```python
from build123d import *

# Parameters (mm, degrees)
BOSS_EXTRUDE1_DEPTH = 80
SKETCH2_R           = 6
CUT_EXTRUDE1_DEPTH  = 12


with BuildPart() as part:
    # Sketch1 → Boss-Extrude1 (new body)
    with BuildSketch(Plane.XY):
        with BuildLine():
            Line((0, 0), (-27, 0))
            ThreePointArc((-27, 0), (-36.192388155, -3.807611845), (-40, -13))
            Line((-40, -13), (-40, -190))
            Line((-40, -190), (-32, -190))
            Line((-32, -190), (-32, -13))
            ThreePointArc((-32, -13), (-30.535533906, -9.464466094), (-27, -8))
            Line((-27, -8), (0, -8))
            Line((0, -8), (0, 0))
        make_face()
    extrude(amount=BOSS_EXTRUDE1_DEPTH)

    # Sketch2 → Cut-Extrude1 (cut)
    with BuildSketch(Plane(origin=(0, 0, 0), x_dir=(1, 0, 0), z_dir=(0, 1, 0))):
        with Locations(Location((-15, -40, 0), (0, 0, 270))):
            Circle(SKETCH2_R)
        Polygon((-20, 0), (0, -30), (0, 0), align=None)
        Polygon((0, -50), (0, -80), (-20, -80), align=None)
    extrude(amount=-CUT_EXTRUDE1_DEPTH, mode=Mode.SUBTRACT)


solid = part.part
```
Geometry check sheet. Reference: the model listing, model coordinates, mm. A direction names the side the tool comes from. Give positions to 0.01 mm unless a question says otherwise; leave off trailing zeros. Loops run counter-clockwise (first coordinate to the right, second up) from the corner with the lowest first, then second, coordinate; pieces in that order, holes last. Notation, with made-up numbers: M 17.25,87 L 32.25,87 A28 ccw 32.25,126 Z; hole C 51,-2 d9. An arc over 180 degrees is marked long. Write item = value, one per line. Start each with the question number.
1. Draft check along X on faces 1 (the face through (-22, 0, 39)), 2 (the face through (-10.94, -3.94, 35.58)), 3 (the face through (-31, -10, 39)). Enter one of: +X half, -X half, draft (parallel to the pull), parting line (faces both ways), or undercut.
2. Thickness scan on probe 1 along Y at (x, z) = (-25, 37); probe 2 along X at (y, z) = (-94, 36.5); probe 3 along X at (y, z) = (-4.75, 40). Record the ranges inside material, lowest first.
3. Go/stop test with flat-tipped pins: P1, Ø8, axis at x = -11.5, z = 34.5, coming from the -Y side; P2, Ø5, axis at y = -49.5, z = 28, coming from the +X side; P3, Ø8, axis at x = -35.5, z = 36, coming from the +Y side. Record where each tip stops, or that it passes through.
4. Section check B-B, the plane x = -15. Enter the section's corners in (y, z).
5. Section check A-A, the plane z = 40. Enter the section's corners in (x, y), plus the area to 3 significant figures.
6. Tool access check on faces 4 (the face through (-10, -4, 15)), 5 (the face through (-23, -8, 39)). Record the directions out of +Z, -Z, +X, -X, +Y, -Y that give a thin tool (end or side, any length) a straight path to the whole face; none if there is none.
7. Section check D-D, the plane y = -87. Enter the section's corners in (x, z).
8. Section check C-C, the plane z = 32. Enter the section's corners in (x, y).
Values follow:
q1.face_1 = draft
q1.face_2 = undercut
q1.face_3 = +X half
q2.probe_1 = -8 to 0
q2.probe_2 = -40 to -32
q2.probe_3 = -37.05 to -21, -9 to 0
q3.P1 = -8
q3.P2 = -32
q3.P3 = -0.8
q4.outline = M -8,7.5 L 0,7.5 L 0,34 L -8,34 Z; M -8,46 L 0,46 L 0,72.5 L -8,72.5 Z
q5.outline = M -40,-190 L -32,-190 L -32,-13 A5 cw -27,-8 L -21,-8 L -21,0 L -27,0 A13 ccw -40,-13 Z; M -9,-8 L 0,-8 L 0,0 L -9,0 Z
q5.area = 1,650 mm^2
q6.face_4 = -Z, +X, +Y, -Y
q6.face_5 = +Z, -Z, +X, -Y
q7.outline = M -40,0 L -32,0 L -32,80 L -40,80 Z
q8.outline = M -40,-190 L -32,-190 L -32,-13 A5 cw -27,-8 L 0,-8 L 0,0 L -27,0 A13 ccw -40,-13 Z
